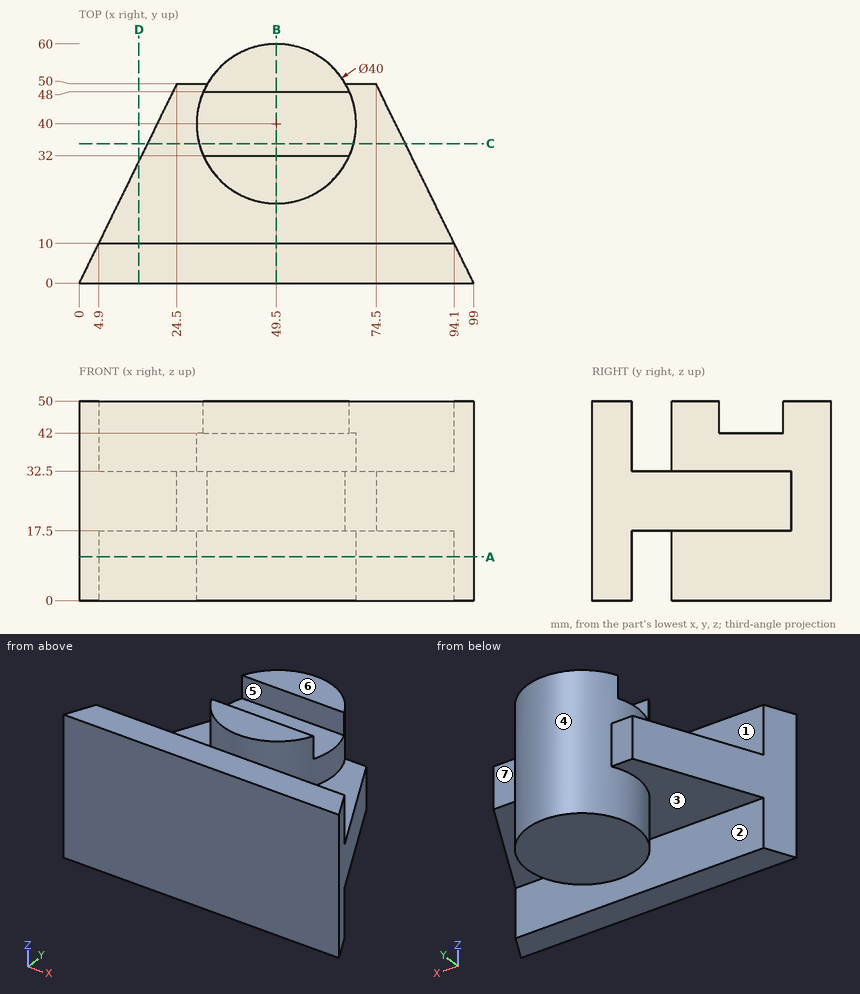
Can you work these out from the drawing? Everything is in mm from the part's minimum corner. A direction names the side the tool comes from. Round coordinates to 2 decimals unless told otherwise and drop trailing zeros. Order: outer loops, then holes, each group sorted by start corner. A loop starts at its lowest first (then second) coordinate and runs counter-clockwise, first axis right, second up. Notation, with made-up numbers: M 28,23 L 57,23 A28 cw 57,53 Z; hole C -7,30 d3. An arc over 180 degrees is marked long. One line per question, with ' | ' between items.
1) I want a section at D-D, the plane x = 15. Write out the boundary of the cut face in (y, z).
Working result:
outline: M 0,0 L 10,0 L 10,17.5 L 30.61,17.5 L 30.61,32.5 L 10,32.5 L 10,50 L 0,50 Z
2) I need wall thicknesses on line 1 along Y through (x, z) = (44, 47); line 2 along Y through (x, z) = (90, 9); line 3 along Z through (x, y) = (34, 40.5). Which ranges of each line are inside material? Lowest first, please.
Working result:
line 1: 0 to 10, 20.77 to 32, 48 to 59.23 | line 2: 0 to 10 | line 3: 0 to 42
3) I want a section at C-C, the plane y = 35. Write out the boundary of the cut face in (x, z), then the cut area to 3 significant figures.
Working result:
outline: M 17.15,17.5 L 30.14,17.5 L 30.14,0 L 68.86,0 L 68.86,17.5 L 81.85,17.5 L 81.85,32.5 L 68.86,32.5 L 68.86,42 L 30.14,42 L 30.14,32.5 L 17.15,32.5 Z | area: 2,020 mm²
4) For pin 1 Ø10 at (x, z) = (32, 39) entering from +Y; pin 2 Ø4 at (x, y) = (76, 52) entering from +Z; pin 3 Ø14 at (x, z) = (42, 41) entering from +Y; pin 4 Ø5 at (x, y) = (37.5, 16) entering from -Z, each with a flat end and sliding along its axis, tell me the tip position at first contact or that it passes through.
Working result:
pin 1: y = 55.61 | pin 2: through | pin 3: y = 59.99 | pin 4: z = 17.5
5) For the marked faces 1, 2, 3 and 4, which set-ups out of +Z, -Z, +X, -X, +Y, -Y let a thin tool reach every point of the face, with its end or its side?
Working result:
face 1: +Z, +X, -X | face 2: -Z, +X, -X | face 3: -Z | face 4: none
6) I want a section at A-A, the plane z = 11. Write out the boundary of the cut face in (x, y).
Working result:
outline: M 0,0 L 99,0 L 94.1,10 L 4.9,10 Z; C 49.5,40 d40
7) I want a section at B-B, the plane x = 49.5. Write out the boundary of the cut face in (y, z).
Working result:
outline: M 0,0 L 10,0 L 10,17.5 L 20,17.5 L 20,0 L 60,0 L 60,50 L 48,50 L 48,42 L 32,42 L 32,50 L 20,50 L 20,32.5 L 10,32.5 L 10,50 L 0,50 Z
8) If we mould it in two halves opening along Y, with no side actions, what happens to the marked faces 5, 6 and 7? For each: +Y half, -Y half, draft (parallel to the pull), parting line (faces both ways), or undercut.
Working result:
face 5: undercut | face 6: draft | face 7: +Y half
